Part model, mm, in its own coordinate system. Face numbers are marked on the shaded views. Give positions to 0.01 mm unless a question says otherwise; leave off trailing zeros. Write each loop counter-clockwise with the first axis right and the second up, starting at its lowest first coordinate (ties: lowest second). Pieces come first, ordered by that corner, then holes. Notation, with made-up numbers: M 55.5,5 L 94.5,5 A24 ccw 94.5,36 Z; hole C -15.75,79.5 d6. An arc over 180 degrees is marked long. Answer as CSV lines item,"result". Start each with the question number.
Item 1: Band-saw the part on B-B, the plane y = -4. List the corners of the cut face in (x, z), then the cut area to 3 significant figures.
Item 2: Band-saw the part on D-D, the plane y = -0.5. List the corners of the cut face in (x, z), then the cut area to 3 significant figures.
Item 3: Pin check, flat tips, straight feed: pin 1 (2 mm diameter, centred on x = -6.5, y = -3.5, fed in from +Z); pin 2 (3 mm diameter, centred on x = 2.5, y = -2, fed in from -Z). Stop position of each tip, or through.
Item 4: Band-saw the part on C-C, the plane y = -5.5. List the corners of the cut face in (x, z), then the cut area to 3 significant figures.
Item 5: Wall check: L1, parallel to Y at x = 0, z = 10.05; L2, parallel to X at y = -3, z = 0; L3, parallel to Z at x = -7, y = -4.25. Give the ranges that are in metal, low to high. Write a range as from..to.
Item 6: Two-plate mould, pull along Z, no slides. Class the marked faces 1, 2 and 3: +Z half, -Z half, draft (parallel to the pull), parting line (faces both ways), or undercut.
Item 7: Band-saw the part on A-A, the plane z = 0. List the corners of the cut face in (x, y), then the cut area to 3 significant figures.
from build123d import *

# Parameters (mm, degrees)
SKETCH1_R               = 12
SKETCH1_R_2             = 8
BOSS_EXTRUDE1_DEPTH     = 8
CUT_EXTRUDE1_DEPTH      = 19.761663039
CUT_EXTRUDE1_DEPTH_BACK = 19.761663039
SKETCH2_R               = 2
FILLET1_R               = 1


with BuildPart() as part:
    # Sketch1 → Boss-Extrude1 (new body)
    with BuildSketch(Plane(origin=(0, 0, 0), x_dir=(1, 0, 0), z_dir=(0, 1, 0))):
        with Locations(Location((0, 0, 0), (0, 0, 270))):
            Circle(SKETCH1_R)
        with Locations(Location((0, 0, 0), (0, 0, 270))):
            Circle(SKETCH1_R_2, mode=Mode.SUBTRACT)
    extrude(amount=-BOSS_EXTRUDE1_DEPTH)

    # Sketch2 → Cut-Extrude1 (cut, two sides: drawn at the far end of the back side and taken through both)
    with BuildSketch(Plane.XY.offset(-CUT_EXTRUDE1_DEPTH_BACK)):
        with Locations((0, -4)):
            Circle(SKETCH2_R)
    extrude(amount=CUT_EXTRUDE1_DEPTH + CUT_EXTRUDE1_DEPTH_BACK, mode=Mode.SUBTRACT)

    # Fillet1
    fillet1_edges = [part.edges().sort_by_distance(p)[0] for p in [
        (0, 0, -12),
    ]]
    fillet(fillet1_edges, radius=FILLET1_R)


solid = part.part
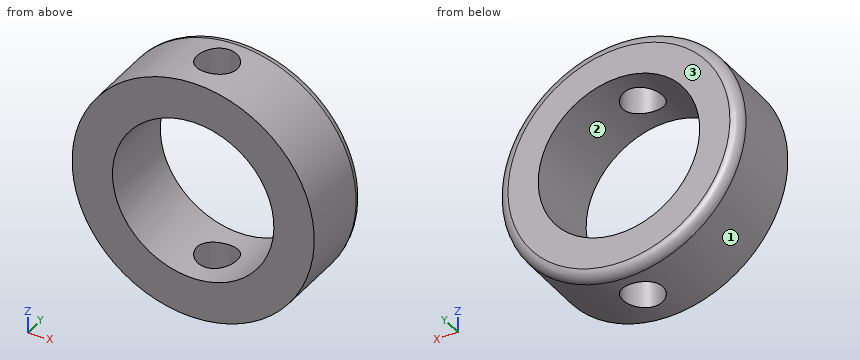
Output:
1,outline,"M -2,-11.83 L -2,-7.75 A8 cw -2,7.75 L -2,11.83 A12 ccw Z; M 2,-11.83 A12 ccw 2,11.83 L 2,7.75 A8 cw 2,-7.75 Z"
1,area,"219 mm²"
2,outline,"C 0,0 d23.73; hole C 0,0 d16"
2,area,"241 mm²"
3,pin 1,"z = 10.67"
3,pin 2,"z = -11.96"
4,outline,"M -1.32,-11.93 L -1.32,-7.89 A8 cw -1.32,7.89 L -1.32,11.93 A12 ccw Z; M 1.32,-11.93 A12 ccw 1.32,11.93 L 1.32,7.89 A8 cw 1.32,-7.89 Z"
4,area,"230 mm²"
5,L1,"-8..-6, -2..0"
5,L2,"-12..-8, 8..12"
5,L3,"-9.75..-3.87, 3.87..9.75"
6,face 1,"parting line"
6,face 2,"undercut"
6,face 3,"draft"
7,outline,"M -12,-8 L -8,-8 L -8,0 L -11,0 A1 ccw -12,-1 Z; M 8,-8 L 12,-8 L 12,-1 A1 ccw 11,0 L 8,0 Z"
7,area,"63.6 mm²"
